from build123d import *

# Parameters (mm, degrees)
EXTRUDE_1_DEPTH               = 10
HOLE_WIZARD_M12_1_D           = 10.2
HOLE_WIZARD_M12_1_CSINK_D     = 12.05
HOLE_WIZARD_M12_1_CSINK_ANGLE = 90


with BuildPart() as part:
    # 草图1 → 凸台-拉伸1 (new body)
    with BuildSketch(Plane.XY):
        with BuildLine():
            Line((-84.801934074, -1426.511579499), (-89.885840943, -1368.402258085))
            ThreePointArc((-89.885840943, -1368.402258085), (-89.971446647, -1367.096167423), (-90, -1365.787585802))
            Line((-90, -1365.787585802), (-90, -632.212414198))
            ThreePointArc((-90, -632.212414198), (-89.971446647, -630.903832577), (-89.885840943, -629.597741915))
            Line((-89.885840943, -629.597741915), (-84.801934074, -571.488420501))
            ThreePointArc((-84.801934074, -571.488420501), (-75.18379936, -551.984772679), (-54.916093131, -544.103092784))
            Line((-54.916093131, -544.103092784), (44.916093131, -544.103092784))
            ThreePointArc((44.916093131, -544.103092784), (65.18379936, -551.984772679), (74.801934074, -571.488420501))
            Line((74.801934074, -571.488420501), (79.885840943, -629.597741915))
            ThreePointArc((79.885840943, -629.597741915), (79.971446647, -630.903832577), (80, -632.212414198))
            Line((80, -632.212414198), (80, -662.212414198))
            ThreePointArc((80, -662.212414198), (75.980762114, -677.212414198), (65, -688.193176311))
            Line((65, -688.193176311), (22, -713.019237886))
            ThreePointArc((22, -713.019237886), (11.019237886, -724), (7, -739))
            Line((7, -739), (7, -1259))
            ThreePointArc((7, -1259), (11.019237886, -1274), (22, -1284.980762114))
            Line((22, -1284.980762114), (65, -1309.806823689))
            ThreePointArc((65, -1309.806823689), (75.980762114, -1320.787585802), (80, -1335.787585802))
            Line((80, -1335.787585802), (80, -1365.787585802))
            ThreePointArc((80, -1365.787585802), (79.971446647, -1367.096167423), (79.885840943, -1368.402258085))
            Line((79.885840943, -1368.402258085), (74.801934074, -1426.511579499))
            ThreePointArc((74.801934074, -1426.511579499), (65.18379936, -1446.015227321), (44.916093131, -1453.896907216))
            Line((44.916093131, -1453.896907216), (-54.916093131, -1453.896907216))
            ThreePointArc((-54.916093131, -1453.896907216), (-75.18379936, -1446.015227321), (-84.801934074, -1426.511579499))
        make_face()
    extrude(amount=EXTRUDE_1_DEPTH)

    # M12 螺纹孔1 (through all)
    with Locations(Plane(origin=(5, -1413.896907216, 10), x_dir=(1, 0, 0), z_dir=(0, 0, 1))):
        with Locations((0, 0), (-40, 0), (-40, 829.793814432), (0, 829.793814432)):
            CounterSinkHole(HOLE_WIZARD_M12_1_D / 2, HOLE_WIZARD_M12_1_CSINK_D / 2, counter_sink_angle=HOLE_WIZARD_M12_1_CSINK_ANGLE)


solid = part.part
Read the model definition and answer for the solid it produces. Units are mm, in the model's axes. A direction names the side the tool comes from. Coordinates: 2 decimals unless noted, no trailing zeros. Loops run counter-clockwise (first coordinate to the right, second up) from the corner with the lowest first, then second, coordinate; pieces in that order, holes last.
Q1. Each of these flat-tipped pins is pushed along its axis until it touches: pin 1 Ø13.5 at (x, y) = (5, -1413.9) entering from +Z; pin 2 Ø5 at (x, z) = (-70.5, 5) entering from -Y; pin 3 Ø9 at (x, y) = (-35, -584.1) entering from +Z. Where does it stop, or does it pass through?
Q2. Consider probe 1 along Y at (x, z) = (-35, 2.5); probe 2 along X at (y, z) = (-1410.5, 2.75); probe 3 along Y at (x, z) = (19, 7.25). Determine where each line is inside the solid, lowest interval first.
Q3. The part is cut by section C-C on y = -1268. Write down the section's boundary in (x, z), and give its area (3 significant figures).
Q4. Which of the six approach directions +Z, -Z, +X, -X, +Y, -Y give full straight-line access (tool end or side, diameter ignored) to faces 4 (the face through (-23, -993, 0)), 5 (the face through (10.91, -1273.81, 4.93))?
Q5. The mould has two halves that part along Y. Classify faces 1 (the face through (64.953, -551.775, 4.93)), 2 (the face through (43.801, -700.432, 4.93)), 3 (the face through (65.412, -1445.804, 4.93)): +Y half, -Y half, draft (parallel to the pull), parting line (faces both ways), or undercut.
Q6. The part is cut by section B-B on y = -820. Write down the section's boundary in (x, z).
Q7. The part is cut by section A-A on z = 5.25. Write down the section's boundary in (x, y), and give its area (3 significant figures).
Results below:
1. pin 1: stops at z = 10
1. pin 2: stops at y = -1450.89
1. pin 3: passes through
2. probe 1: y = -1453.9 to -1419, -1408.8 to -589.2, -579 to -544.1
2. probe 2: x = -86.2 to -38.8, -31.2 to 1.2, 8.8 to 76.2
2. probe 3: y = -1453.9 to -1283, -715 to -544.1
3. outline: (-90, 0) - (8.38, 0) - (8.38, 10) - (-90, 10) - close
3. area: 984 mm2
4. face 4: -Z, +X, -X, +Y, -Y
4. face 5: +Z, -Z, +X
5. face 1: +Y half
5. face 2: undercut
5. face 3: -Y half
6. outline: (-90, 0) - (7, 0) - (7, 10) - (-90, 10) - close
7. outline: (-90, -1365.79) arc R30 ccw to (-89.89, -1368.4) - (-84.8, -1426.51) arc R30 ccw to (-54.92, -1453.9) - (44.92, -1453.9) arc R30 ccw to (74.8, -1426.51) - (79.89, -1368.4) arc R30 ccw to (80, -1365.79) - (80, -1335.79) arc R30 ccw to (65, -1309.81) - (22, -1284.98) arc R30 cw to (7, -1259) - (7, -739) arc R30 cw to (22, -713.02) - (65, -688.19) arc R30 ccw to (80, -662.21) - (80, -632.21) arc R30 ccw to (79.89, -629.6) - (74.8, -571.49) arc R30 ccw to (44.92, -544.1) - (-54.92, -544.1) arc R30 ccw to (-84.8, -571.49) - (-89.89, -629.6) arc R30 ccw to (-90, -632.21) - close; hole circle Ø10.2 at (-35, -1413.9); hole circle Ø10.2 at (-35, -584.1); hole circle Ø10.2 at (5, -1413.9); hole circle Ø10.2 at (5, -584.1)
7. area: 109,000 mm2
